Here's how the part is built. I have some questions about the finished solid (model axes, mm). A direction names the side the tool comes from. Coordinates: 2 decimals unless noted, no trailing zeros. Loops run counter-clockwise (first coordinate to the right, second up) from the corner with the lowest first, then second, coordinate; pieces in that order, holes last.
from build123d import *

# Parameters (mm, degrees)
SKETCH1_R           = 3.5
BASEHEAD_DEPTH      = 4
SKETCH2_R           = 2
BASEBODY_DEPTH      = 20
HEXAGONSOCKET_DEPTH = 2
TOPFILLET_R         = 0.5
CHAMFER1_SIZE       = 0.2


with BuildPart() as part:
    # Sketch1 → BaseHead (new body)
    with BuildSketch(Plane(origin=(0, 0, 0), x_dir=(0, 0, -1), z_dir=(1, 0, 0))):
        Circle(SKETCH1_R)
    extrude(amount=BASEHEAD_DEPTH)

    # Sketch2 → BaseBody (add)
    with BuildSketch(Plane(origin=(4, 0, 0), x_dir=(0, 0, -1), z_dir=(1, 0, 0))):
        Circle(SKETCH2_R)
    extrude(amount=BASEBODY_DEPTH)

    # Sketch3 → HexagonSocket (cut)
    with BuildSketch(Plane(origin=(0, 0, 0), x_dir=(0, 0, -1), z_dir=(1, 0, 0))):
        Polygon((1.732050808, 0), (0.866025404, 1.5), (-0.866025404, 1.5), (-1.732050808, 0), (-0.866025404, -1.5), (0.866025404, -1.5), align=None)
    extrude(amount=HEXAGONSOCKET_DEPTH, mode=Mode.SUBTRACT)

    # Sketch4 → Cut-Revolve1 (revolve, cut)
    with BuildSketch(Plane(origin=(-4.19613823, 0.75, 0), x_dir=(-1, 0, 0), z_dir=(0, 0, 1)), mode=Mode.PRIVATE) as cut_revolve1_sk:
        Polygon((-6.19613823, 2.25), (-7.062163633, 0.75), (-6.19613823, 0.75), align=None)
    revolve(cut_revolve1_sk.sketch.rotate(Axis((0.838992387, 0, 0), (-1, 0, 0)), 90), axis=Axis((0.838992387, 0, 0), (-1, 0, 0)), mode=Mode.SUBTRACT)

    # TopFillet
    topfillet_edges = [part.edges().sort_by_distance(p)[0] for p in [
        (0, 0, 3.5),
    ]]
    fillet(topfillet_edges, radius=TOPFILLET_R)

    # Chamfer1
    chamfer1_edges = [part.edges().sort_by_distance(p)[0] for p in [
        (24, 0, 2),
    ]]
    chamfer(chamfer1_edges, length=CHAMFER1_SIZE)


solid = part.part
Q1. We'd pull the mould along Z, two halves only. Please class faces 1 (the flat face through (4, -2, -2)), 2 (the flat face through (0.986, 0.74, -1.305)), 3 (the cylindrical face through (2.226, -1.341, -3.233)), 4 (the flat face through (0.986, 0.76, 1.293)): pulls with the +Z half, pulls with the -Z half, needs draft (parallel to the pull), parting line crosses it, or undercut.
Q2. Suppose I cut it at A-A on x = 1.75. Write out the boundary of the cut face in (y, z), and give its area (3 significant figures).
Q3. Please list where these lines run through material, in increasing order: probe 1 along X at (y, z) = (0.5, -3); probe 2 along Y at (x, z) = (13.25, 0); probe 3 along X at (y, z) = (-1, -1.5).
Q4. Suppose I cut it at B-B on x = 15.5. Write out the boundary of the cut face in (y, z).
Q5. Will these pins go through, and if not, where does the flat tip stop? P1, Ø3, axis at x = 14, y = 1, coming from the +Z side; P2, Ø4, axis at x = 19, z = -0.5, coming from the -Y side; P3, Ø0.6, axis at y = -1, z = 0.5, coming from the -X side; P4, Ø0.5, axis at y = 0, z = 1.5, coming from the -X side.
Q6. For faces 5 (the flat face through (1, 1.5, 0)), 6 (the cylindrical face through (14, -2, 0)), 7 (the flat face through (24, 0, 0)), which set-ups out of +Z, -Z, +X, -X, +Y, -Y let a thin tool reach every point of the face, with its end or its side?
Check values:
1. face 1: needs draft
1. face 2: undercut
1. face 3: parting line crosses it
1. face 4: undercut
2. outline: circle Ø7 at (0, 0); hole (-1.5, -0.87) - (0, -1.73) - (1.5, -0.87) - (1.5, 0.87) - (0, 1.73) - (-1.5, 0.87) - close
2. area: 30.7 mm2
3. probe 1: x = 0 to 4
3. probe 2: y = -2 to 2
3. probe 3: x = 0 to 24
4. outline: circle Ø4 at (0, 0)
5. P1: stops at z = 2
5. P2: stops at y = -2
5. P3: stops at x = 2.05
5. P4: stops at x = 0
6. face 5: -X
6. face 6: +X
6. face 7: +Z, -Z, +X, +Y, -Y
